Input: part model. Units: mm. Frame: model coordinates. Face numbers are marked on the shaded views. A direction names the side the tool comes from. Coordinates: 2 decimals unless noted, no trailing zeros. Order: outer loops, then holes, each group sorted by start corner. A loop starts at its lowest first (then second) coordinate and runs counter-clockwise, first axis right, second up. Notation, with made-up numbers: (-20.5, -22.5) - (-13.5, -22.5) arc R22 cw to (-13.5, 0.5) - close; hole circle Ø9 at (75, 37). An arc over 180 degrees is marked (long way). One line per question, with ' | ' between items.
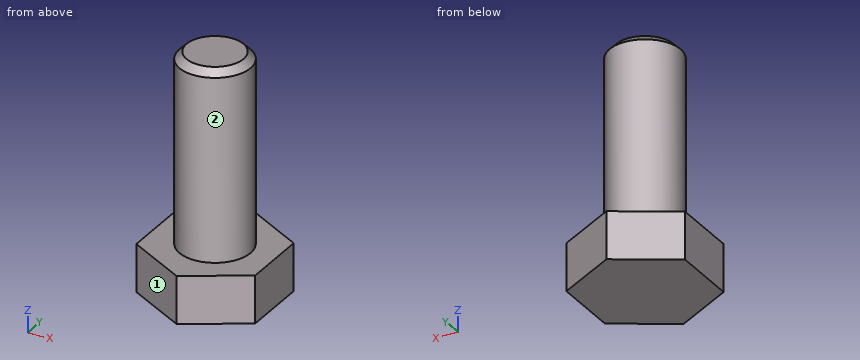
from build123d import *

# Parameters (mm, degrees)
BOSS_EXTRUDE1_DEPTH = 4
SKETCH3_R           = 3
BOSS_EXTRUDE2_DEPTH = 16
CHAMFER1_SIZE       = 0.6


with BuildPart() as part:
    # Sketch1 → Boss-Extrude1 (new body)
    with BuildSketch(Plane.XY):
        Polygon((5, 2.886751346), (0, 5.773502692), (-5, 2.886751346), (-5, -2.886751346), (0, -5.773502692), (5, -2.886751346), align=None)
    extrude(amount=BOSS_EXTRUDE1_DEPTH)

    # Sketch3 → Boss-Extrude2 (add)
    with BuildSketch(Plane.XY.offset(4)):
        Circle(SKETCH3_R)
    extrude(amount=BOSS_EXTRUDE2_DEPTH)

    # Chamfer1
    chamfer1_edges = [part.edges().sort_by_distance(p)[0] for p in [
        (-3, 0, 20),
    ]]
    chamfer(chamfer1_edges, length=CHAMFER1_SIZE)


solid = part.part
Item 1: Section D-D on z = 14.25. Return the cut outline in (x, y).
Data:
outline: circle Ø6 at (0, 0)
Item 2: Contact query for flat-ended pins moving along their axis: P1, Ø6, axis at y = -3, z = 11, coming from the +X side; P2, Ø5, axis at x = -1, z = 18, coming from the +Y side; P3, Ø3, axis at y = 2, z = 8.5, coming from the -X side. Output: stop coordinate, or through.
Data:
P1: x = 3 | P2: y = 3 | P3: x = -2.96
Item 3: Section A-A on y = 0. Return the cut outline in (x, z), and give its area (3 significant figures).
Data:
outline: (-5, 0) - (5, 0) - (5, 4) - (3, 4) - (3, 19.4) - (2.4, 20) - (-2.4, 20) - (-3, 19.4) - (-3, 4) - (-5, 4) - close | area: 136 mm^2
Item 4: Access query for the marked faces 1 and 2. Directions: +Z, -Z, +X, -X, +Y, -Y. A direction counts if a zero-diameter tool reaches every point of the face in a straight line with its end or side. Return the directions, or none.
Data:
face 1: +Z, -Z, -X, -Y | face 2: +Z
Item 5: Section B-B on z = 1.75. Return the cut outline in (x, y), and give its area (3 significant figures).
Data:
outline: (-5, -2.89) - (0, -5.77) - (5, -2.89) - (5, 2.89) - (0, 5.77) - (-5, 2.89) - close | area: 86.6 mm^2
Item 6: Ray query, line 1 (Z direction, x = 4.25, y = -2.25); line 2 (Y direction, x = 1, z = 15.75); line 3 (Z direction, x = -2, y = 1.75). Return the intervals inside material, ascending.
Data:
line 1: 0 to 4 | line 2: -2.83 to 2.83 | line 3: 0 to 19.74
Item 7: Section C-C on x = -3.5. Return the cut outline in (y, z).
Data:
outline: (-3.75, 0) - (3.75, 0) - (3.75, 4) - (-3.75, 4) - close
